```python
from build123d import *

# Parameters (mm, degrees)
SKETCH2_R           = 0.4
BOSS_EXTRUDE1_DEPTH = 0.5
SKETCH4_R           = 1
SKETCH4_R_2         = 0.5
CUT_EXTRUDE3_DEPTH  = 6
SKETCH5_R           = 0.15
CUT_EXTRUDE4_DEPTH  = 10


with BuildPart() as part:
    # Sketch1 → Revolve1 (revolve)
    with BuildSketch(Plane.XY, mode=Mode.PRIVATE) as revolve1_sk:
        Polygon((0, 0), (0, 1.5), (1, 1.5), (1, 1), (7, 1), (7, 0), align=None)
    revolve(revolve1_sk.sketch.rotate(Axis((0.124352332, 0, 0), (1, 0, 0)), 90), axis=Axis((0.124352332, 0, 0), (1, 0, 0)))

    # Sketch2 → Boss-Extrude1 (add, symmetric)
    with BuildSketch(Plane.XY):
        with BuildLine():
            Line((0, 0.75), (0, -0.75))
            Line((0, -0.75), (-3, -0.75))
            ThreePointArc((-3, -0.75), (-3.75, 0), (-3, 0.75))
            Line((-3, 0.75), (0, 0.75))
        make_face()
        with Locations((-3, 0)):
            Circle(SKETCH2_R, mode=Mode.SUBTRACT)
    extrude(amount=BOSS_EXTRUDE1_DEPTH, both=True)

    # Sketch4 → Cut-Extrude3 (cut)
    with BuildSketch(Plane(origin=(7, 0, 0), x_dir=(0, 0, -1), z_dir=(1, 0, 0))):
        Circle(SKETCH4_R)
        Circle(SKETCH4_R_2, mode=Mode.SUBTRACT)
    extrude(amount=-CUT_EXTRUDE3_DEPTH, mode=Mode.SUBTRACT)

    # Sketch5 → Cut-Extrude4 (cut)
    with BuildSketch(Plane.ZY):
        with Locations((0.7, 0)):
            Circle(SKETCH5_R)
    extrude(amount=-CUT_EXTRUDE4_DEPTH, mode=Mode.SUBTRACT)


solid = part.part
```
Geometry: final body of the model. Coordinates: model frame, mm. A direction names the side the tool comes from. Coordinates: 2 decimals unless noted, no trailing zeros. Order: outer loops, then holes, each group sorted by start corner. A loop starts at its lowest first (then second) coordinate and runs counter-clockwise, first axis right, second up. Notation, with made-up numbers: (48, 39.25) - (88, 39.25) arc R29 cw to (88, 68.25) - close; hole circle Ø9 at (45.5, 42). An arc over 180 degrees is marked (long way). Write each question's results on one line, items separated by ' | '.
(1) Section query D-D, the plane y = 1.2. Return the cut outline in (x, z), plus the area to 3 significant figures.
Values found:
outline: (0, -0.9) - (1, -0.9) - (1, 0.9) - (0, 0.9) - close | area: 1.80 mm²
(2) Section query A-A, the plane y = 0. Return the cut outline in (x, z), plus the area to 4 significant figures.
Values found:
outline: (-3.75, -0.5) - (-3.4, -0.5) - (-3.4, 0.5) - (-3.75, 0.5) - close; (-2.6, -0.5) - (0, -0.5) - (0, -1.5) - (1, -1.5) - (1, -0.5) - (7, -0.5) - (7, 0.5) - (1, 0.5) - (1, 0.55) - (0, 0.55) - (0, 0.5) - (-2.6, 0.5) - close; (0, 0.85) - (1, 0.85) - (1, 1.5) - (0, 1.5) - close | area: 11.65 mm²
(3) First-contact query: pin 1 Ø1 at (x, z) = (-1.5, -0.5) entering from -Y; pin 2 Ø1.5 at (y, z) = (0.5, -1) entering from +X; pin 3 Ø0.5 at (x, z) = (-2, 0) entering from +Y. Flat tips, straight axial feed; report the tip coordinate or a pass-through.
Values found:
pin 1: stops at y = -0.75 | pin 2: stops at x = 7 | pin 3: stops at y = 0.75
(4) Set-up query: faces 1 (the face through (1, 1, 0)), 2 (the face through (-2, 0.75, 0)), 3 (the face through (-2, 0, 0.5)), 4 (the face through (-1, -0.75, 0)), 5 (the face through (-2, 0, -0.5)). Return all of +Z, -Z, +X, -X, +Y, -Y with unobstructed straight access to the full face (end or side cutting, diameter ignored); none if empty.
Values found:
face 1: +X | face 2: +Z, -Z, -X, +Y | face 3: +Z, -X, +Y, -Y | face 4: +Z, -Z, -X, -Y | face 5: -Z, -X, +Y, -Y
(5) Section query B-B, the plane z = 0.7. Return the cut outline in (x, y).
Values found:
outline: (0, -1.33) - (1, -1.33) - (1, -0.15) - (0, -0.15) - close; (0, 0.15) - (1, 0.15) - (1, 1.33) - (0, 1.33) - close
(6) Line query: line 1 (Z direction, x = -1.75, y = 0.3); line 2 (X direction, y = -0.35, z = 1.15); line 3 (Y direction, x = 3.5, z = -0.4). Output: solid intervals per line, ascending. Write a range as [from, to].
Values found:
line 1: z = [-0.5, 0.5] | line 2: x = [0, 1] | line 3: y = [-0.3, 0.3]
(7) Section query C-C, the plane x = 3.75. Return the cut outline in (y, z).
Values found:
outline: circle Ø1 at (0, 0)
